```python
from build123d import *

# Parameters (mm, degrees)
BASE_PLATE_SKETCH_W       = 106
BASE_PLATE_SKETCH_H       = 82
BASE_PLATE_DEPTH          = 12
UPRIGHT_WALL_SKETCH_W     = 10
UPRIGHT_WALL_SKETCH_H     = 34
UPRIGHT_WALL_DEPTH        = 82
WALL_ROOT_FILLET_R12_R    = 12
MOUNTING_LUG_1_SKETCH_W   = 82
MOUNTING_LUG_1_SKETCH_H   = 24
MOUNTING_LUG_1_DEPTH      = 12
LUG_1_CORNER_FILLET_R12_R = 12
LUG_1_HOLE_SKETCH_R       = 5
LUG_1_MOUNTING_HOLE_DEPTH = 123.609135059
MOUNTING_LUG_2_SKETCH_W   = 82
MOUNTING_LUG_2_SKETCH_H   = 24
MOUNTING_LUG_2_DEPTH      = 12
LUG_2_CORNER_FILLET_R12_R = 12
LUG_START                 = -12
LUG_2_HOLE_SKETCH_R       = 5
LUG_2_MOUNTING_HOLE_DEPTH = 12
SIDE_SUPPORT_DEPTH        = 6
GROOVED_CLAMP_RAIL_DEPTH  = 82


with BuildPart() as part:
    # Base Plate Sketch → Base Plate (new body)
    with BuildSketch(Plane(origin=(0, 0, 0), x_dir=(1, 0, 0), z_dir=(0, 1, 0))):
        Rectangle(BASE_PLATE_SKETCH_W, BASE_PLATE_SKETCH_H)
    extrude(amount=BASE_PLATE_DEPTH)

    # Upright Wall Sketch → Upright Wall (add)
    with BuildSketch(Plane.XY.offset(41)):
        with Locations((48, 29)):
            Rectangle(UPRIGHT_WALL_SKETCH_W, UPRIGHT_WALL_SKETCH_H)
    extrude(amount=-UPRIGHT_WALL_DEPTH)

    # Wall Root Fillet R12
    wall_root_fillet_r12_edges = [part.edges().sort_by_distance(p)[0] for p in [
        (43, 12, 0),
    ]]
    fillet(wall_root_fillet_r12_edges, radius=WALL_ROOT_FILLET_R12_R)

    # Mounting Lug 1 Sketch → Mounting Lug 1 (add)
    with BuildSketch(Plane.ZY.offset(53)):
        with Locations((0, -12)):
            Rectangle(MOUNTING_LUG_1_SKETCH_W, MOUNTING_LUG_1_SKETCH_H)
    extrude(amount=-MOUNTING_LUG_1_DEPTH)

    # Lug 1 Corner Fillet R12
    lug_1_corner_fillet_r12_edges = [part.edges().sort_by_distance(p)[0] for p in [
        (-47, -24, -41),
        (-47, -24, 41),
    ]]
    fillet(lug_1_corner_fillet_r12_edges, radius=LUG_1_CORNER_FILLET_R12_R)

    # Lug 1 Hole Sketch → Lug 1 Mounting Hole (cut, through all)
    with BuildSketch(Plane.ZY.offset(53)):
        with Locations((-29, -12)):
            Circle(LUG_1_HOLE_SKETCH_R)
        with Locations((29, -12)):
            Circle(LUG_1_HOLE_SKETCH_R)
    extrude(amount=-LUG_1_MOUNTING_HOLE_DEPTH, mode=Mode.SUBTRACT)

    # Mounting Lug 2 Sketch → Mounting Lug 2 (add)
    with BuildSketch(Plane(origin=(53, 0, 0), x_dir=(0, 0, -1), z_dir=(1, 0, 0))):
        with Locations((0, -12)):
            Rectangle(MOUNTING_LUG_2_SKETCH_W, MOUNTING_LUG_2_SKETCH_H)
    extrude(amount=-MOUNTING_LUG_2_DEPTH)

    # Lug 2 Corner Fillet R12
    lug_2_corner_fillet_r12_edges = [part.edges().sort_by_distance(p)[0] for p in [
        (47, -24, 41),
        (47, -24, -41),
    ]]
    fillet(lug_2_corner_fillet_r12_edges, radius=LUG_2_CORNER_FILLET_R12_R)

    # Lug 2 Hole Sketch → Lug 2 Mounting Hole (cut)
    with BuildSketch(Plane(origin=(53, 0, 0), x_dir=(0, 0, -1), z_dir=(1, 0, 0)).offset(LUG_START)):
        with Locations(Location((-29, -12, 0), (0, 0, 180))):
            Circle(LUG_2_HOLE_SKETCH_R)
        with Locations(Location((29, -12, 0), (0, 0, 180))):
            Circle(LUG_2_HOLE_SKETCH_R)
    extrude(amount=LUG_2_MOUNTING_HOLE_DEPTH, mode=Mode.SUBTRACT)

    # Side Support Sketch → Side Support (add, symmetric)
    with BuildSketch(Plane.XY):
        with BuildLine():
            Line((-53, 12), (43, 46))
            Line((43, 46), (43, 24))
            ThreePointArc((43, 24), (39.485281374, 15.514718626), (31, 12))
            Line((31, 12), (-53, 12))
        make_face()
    extrude(amount=SIDE_SUPPORT_DEPTH, both=True)

    # Clamp Rail Profile Sketch → Grooved Clamp Rail (add)
    with BuildSketch(Plane.XY.offset(41)):
        with BuildLine():
            Line((53, 46), (55, 46))
            ThreePointArc((55, 46), (65, 36), (75, 46))
            Line((75, 46), (87, 46))
            ThreePointArc((87, 46), (80.583221155, 30.470569282), (65.076071052, 24.000131519))
            ThreePointArc((65.076071052, 24.000131519), (58.103421188, 22.112388202), (53, 17))
            Line((53, 17), (53, 46))
        make_face()
    extrude(amount=-GROOVED_CLAMP_RAIL_DEPTH)


solid = part.part
```
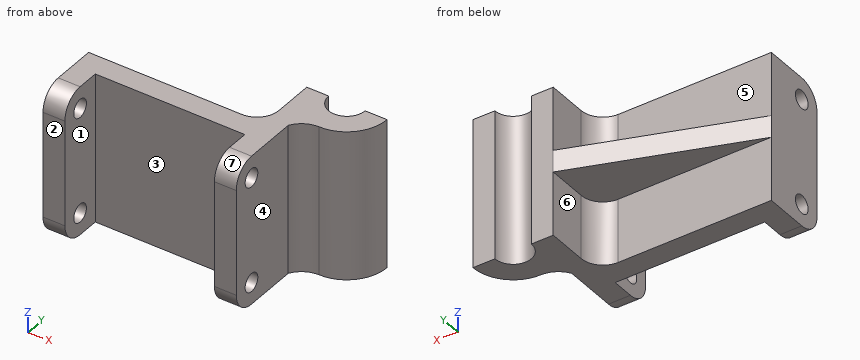
Design review of the part built by this model. Coordinates are the model's own, in mm. Face numbers are marked on the shaded views. A direction names the side the tool comes from. Coordinates: 2 decimals unless noted, no trailing zeros. Loops run counter-clockwise (first coordinate to the right, second up) from the corner with the lowest first, then second, coordinate; pieces in that order, holes last.
Q1. We need section D-D on z = 36. State the section outline as (x, y) points.
Reported:
outline: (-53, -21.75) - (-41, -21.75) - (-41, 0) - (41, 0) - (41, -21.75) - (53, -21.75) - (53, 17) arc R14 cw to (65.08, 24) arc R22 ccw to (87, 46) - (75, 46) arc R10 cw to (55, 46) - (43, 46) - (43, 24) arc R12 cw to (31, 12) - (-53, 12) - close
Q2. Tool access review of the marked faces 5, 6 and 7: name each direction out of +Z, -Z, +X, -X, +Y, -Y from which nothing blocks a thin tool from reaching the whole face with its end or side.
Reported:
face 5: +Z, -X, +Y
face 6: -Z, -X, +Y
face 7: +Z, +X, -X, -Y
Q3. To check wall thickness, follow line 1 (Z direction, x = 47, y = -12); line 2 (X direction, y = -7.5, z = 13); line 3 (Y direction, x = -49, z = 29). State the ranges of each line that lie inside material, in increasing order.
Reported:
line 1: z = -41 to -34, -24 to 24, 34 to 41
line 2: x = -53 to -41, 41 to 53
line 3: y = -24 to -17, -7 to 12
Q4. We need section A-A on z = 0. State the section outline as (x, y) points.
Reported:
outline: (-53, -24) - (-41, -24) - (-41, 0) - (41, 0) - (41, -24) - (53, -24) - (53, 17) arc R14 cw to (65.08, 24) arc R22 ccw to (87, 46) - (75, 46) arc R10 cw to (55, 46) - (43, 46) - (-53, 12) - close
Q5. For pin 1 (13 mm diameter, centred on y = -12, z = 29, fed in from +X); pin 2 (10 mm diameter, centred on x = -11, y = 23.5, fed in from -Z); pin 3 (11 mm diameter, centred on y = 40, z = -21.5, fed in from -X), all flat-tipped, find the tip position at first contact; note any pin that passes through.
Reported:
pin 1: stops at x = 53
pin 2: stops at z = -6
pin 3: stops at x = 43
Q6. We need section C-C on x = 5. State the section outline as (y, z) points, and give its area (3 significant figures).
Reported:
outline: (0, -41) - (12, -41) - (12, -6) - (32.54, -6) - (32.54, 6) - (12, 6) - (12, 41) - (0, 41) - close
area: 1,230 mm2
Q7. The part is to be moulded in two halves that separate along X. For the marked faces 1, 2, 3 and 4, say which applies: +X half, -X half, draft (parallel to the pull), parting line (faces both ways), or undercut.
Reported:
face 1: undercut
face 2: draft
face 3: undercut
face 4: +X half
Q8. We need section B-B on y = 15. State the section outline as (x, z) points.
Reported:
outline: (-44.53, -6) - (38.94, -6) - (38.94, -41) - (53, -41) - (53, 41) - (38.94, 41) - (38.94, 6) - (-44.53, 6) - close
